Can you work these out from the drawing? Everything is in mm from the part's minimum corner. Round coordinates to 2 decimals unless told otherwise and drop trailing zeros. Loops run counter-clockwise (first coordinate to the right, second up) from the corner with the lowest first, then second, coordinate; pieces in that order, holes last. Notation, with made-up numbers: (35, 27) -> (89, 27) arc R8 ccw to (89, 32) -> close; hole circle Ø2 at (53.5, 56.25). An arc over 180 degrees is marked (long way). Answer as a JSON object with one key per item and string values.
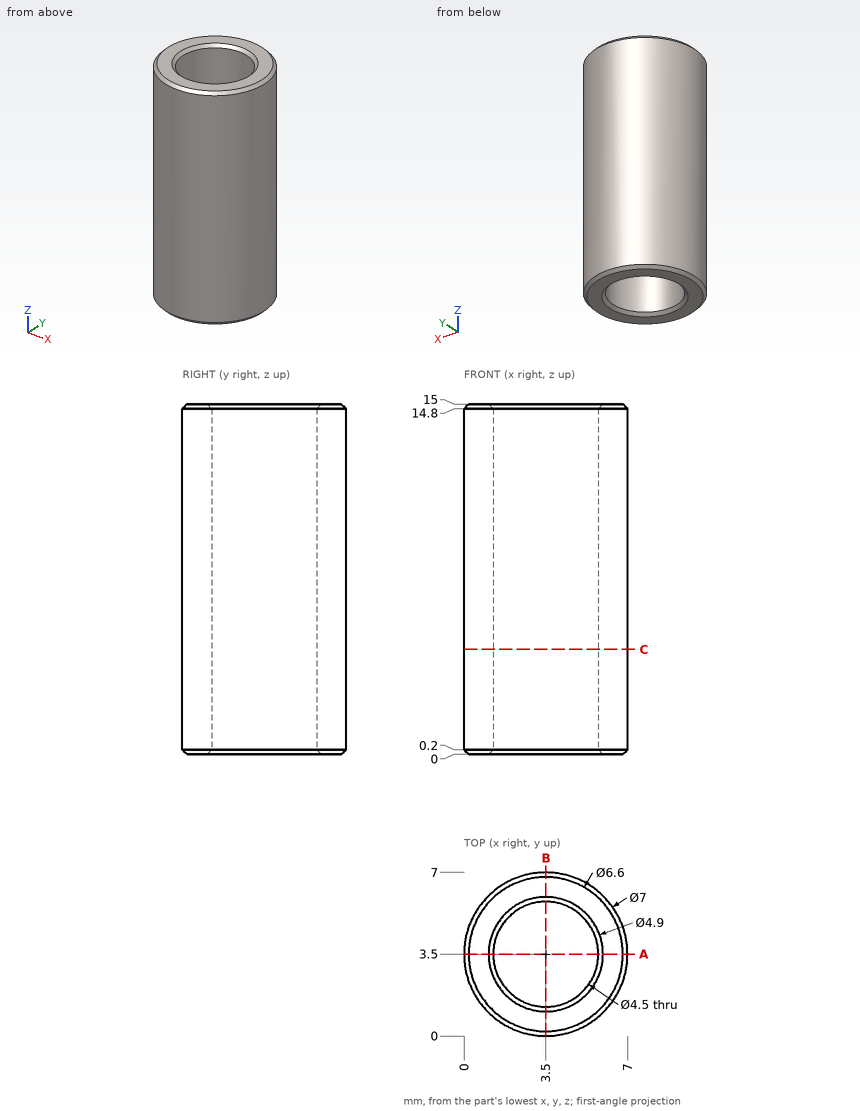
Q1. I'm going to push flat-ended pins straight in: pin 1 (2 mm diameter, centred on y = 2, z = 9, fed in from +X); pin 2 (4 mm diameter, centred on x = 6, z = 9, fed in from -Y); pin 3 (1.5 mm diameter, centred on x = 1.5, z = 12, fed in from +Y). Where does each tip first touch, or does it pass through?
Determined:
{"pin 1": "x = 6.96", "pin 2": "y = 0.04", "pin 3": "y = 6.77"}
Q2. I want a section at A-A, the plane y = 3.5. Write out the boundary of the cut face in (x, z).
Determined:
{"outline": "(0, 0.2) -> (0.2, 0) -> (1.05, 0) -> (1.25, 0.2) -> (1.25, 14.8) -> (1.05, 15) -> (0.2, 15) -> (0, 14.8) -> close; (5.75, 0.2) -> (5.95, 0) -> (6.8, 0) -> (7, 0.2) -> (7, 14.8) -> (6.8, 15) -> (5.95, 15) -> (5.75, 14.8) -> close"}
Q3. If I drill on L1, parallel to Y at x = 3.5, z = 8.75; L2, parallel to Y at x = 4.5, z = 10; L3, parallel to X at y = 1, z = 4.25, over which ranges is the centre line in solid material (lowest first)? Write a range as [from, to].
Determined:
{"L1": "[0, 1.25], [5.75, 7]", "L2": "[0.15, 1.48], [5.52, 6.85]", "L3": "[1.05, 5.95]"}
Q4. I want a section at C-C, the plane z = 4.5. Write out the boundary of the cut face in (x, y).
Determined:
{"outline": "circle Ø7 at (3.5, 3.5); hole circle Ø4.5 at (3.5, 3.5)"}
